Design review of the part built by this model. Coordinates are the model's own, in mm. Face numbers are marked on the shaded views. A direction names the side the tool comes from. Give positions to 0.01 mm unless a question says otherwise; leave off trailing zeros. Write each loop counter-clockwise with the first axis right and the second up, starting at its lowest first coordinate (ties: lowest second). Pieces come first, ordered by that corner, then holes. Notation, with made-up numbers: (73.25, 37) -> (130.25, 37) arc R15 ccw to (130.25, 62) -> close; hole circle Ø9 at (2, 45). An arc over 180 degrees is marked (long way). Answer as a JSON object with one key per item and string values.
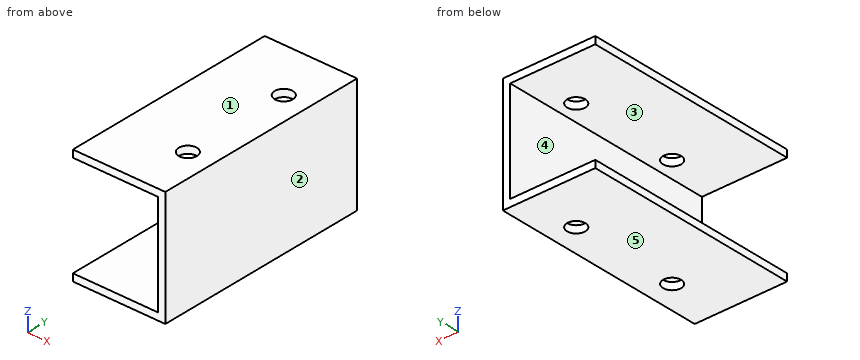
```python
from build123d import *

# Parameters (mm, degrees)
BOSS_EXTRUDE1_DEPTH      = 30
BOSS_EXTRUDE1_DEPTH_BACK = 30
SKETCH3_R                = 2.5
CUT_EXTRUDE1_DEPTH       = 96.420123664


with BuildPart() as part:
    # Sketch2 → Boss-Extrude1 (new, two sides: drawn at the far end of the back side and taken through both)
    with BuildSketch(Plane(origin=(0, 50, 0), x_dir=(-1, 0, 0), z_dir=(0, -1, 0)).offset(-BOSS_EXTRUDE1_DEPTH_BACK)):
        Polygon((-39, 28), (-15.526318688, 28), (-15.526318688, 30), (-41, 30), (-41, -2), (-15.526318688, -2), (-15.526318688, 0), (-39, 0), align=None)
    extrude(amount=BOSS_EXTRUDE1_DEPTH + BOSS_EXTRUDE1_DEPTH_BACK)

    # Sketch3 → Cut-Extrude1 (cut, symmetric)
    with BuildSketch(Plane.XY.offset(2)):
        with Locations((34, 65)):
            Circle(SKETCH3_R)
    cut_extrude1 = extrude(amount=CUT_EXTRUDE1_DEPTH, both=True, mode=Mode.SUBTRACT)

    # Mirror1: Cut-Extrude1 across plane
    add(cut_extrude1.mirror(Plane(origin=(0, 50, 0), x_dir=(0, 0, 1), z_dir=(0, -1, 0))), mode=Mode.SUBTRACT)


solid = part.part
```
(1) The part is to be moulded in two halves that separate along Z. For the marked faces 1, 2 and 3, say which applies: +Z half, -Z half, draft (parallel to the pull), parting line (faces both ways), or undercut.
Here are the results:
{"face 1": "+Z half", "face 2": "draft", "face 3": "undercut"}
(2) We need section C-C, the plane x = 25.75. State the section outline as (y, z) points.
Here are the results:
{"outline": "(20, -30) -> (80, -30) -> (80, -28) -> (20, -28) -> close; (20, 0) -> (80, 0) -> (80, 2) -> (20, 2) -> close"}
(3) For the marked faces 4 and 5, list the 3-axis set-ups (+Z, -Z, +X, -X, +Y, -Y) from which the entire face can be reached by the end or side of a thin tool; tool diameter is ignored.
Here are the results:
{"face 4": "-X, +Y, -Y", "face 5": "-Z, +X, -X, +Y, -Y"}
(4) We need section B-B, the plane y = 65. State the section outline as (x, z) points.
Here are the results:
{"outline": "(15.53, -30) -> (31.5, -30) -> (31.5, -28) -> (15.53, -28) -> close; (15.53, 0) -> (31.5, 0) -> (31.5, 2) -> (15.53, 2) -> close; (36.5, -30) -> (41, -30) -> (41, 2) -> (36.5, 2) -> (36.5, 0) -> (39, 0) -> (39, -28) -> (36.5, -28) -> close"}
(5) We need section A-A, the plane x = 35.5. State the section outline as (y, z) points, then the cut area to 3 significant figures.
Here are the results:
{"outline": "(20, -30) -> (33, -30) -> (33, -28) -> (20, -28) -> close; (20, 0) -> (33, 0) -> (33, 2) -> (20, 2) -> close; (37, -30) -> (63, -30) -> (63, -28) -> (37, -28) -> close; (37, 0) -> (63, 0) -> (63, 2) -> (37, 2) -> close; (67, -30) -> (80, -30) -> (80, -28) -> (67, -28) -> close; (67, 0) -> (80, 0) -> (80, 2) -> (67, 2) -> close", "area": "208 mm²"}
(6) For line 1 along Y through (x, z) = (34, -28.5); line 2 along Z through (x, y) = (37.5, 73); line 3 along X through (y, z) = (43.5, -26.5), list the stretches that pass through material, from the lowest coordinate up.
Here are the results:
{"line 1": "y = 20 to 32.5, 37.5 to 62.5, 67.5 to 80", "line 2": "z = -30 to -28, 0 to 2", "line 3": "x = 39 to 41"}
(7) We need section D-D, the plane y = 54. State the section outline as (x, z) points.
Here are the results:
{"outline": "(15.53, -30) -> (41, -30) -> (41, 2) -> (15.53, 2) -> (15.53, 0) -> (39, 0) -> (39, -28) -> (15.53, -28) -> close"}
